Design review of the part built by this model. Coordinates are the model's own, in mm. Give positions to 0.01 mm unless a question says otherwise; leave off trailing zeros. Write each loop counter-clockwise with the first axis right and the second up, starting at its lowest first coordinate (ties: lowest second). Pieces come first, ordered by that corner, then holes. Notation, with made-up numbers: M 38,47.25 L 60,47.25 A18 cw 60,74.25 Z; hole C -24,54.25 d3. An arc over 180 degrees is marked long. Answer in a Markdown table with one row per item.
```python
from build123d import *

# Parameters (mm, degrees)
SKETCH1_W                      = 128
SKETCH1_H                      = 90
BOSS_EXTRUDE1_DEPTH            = 30
SKETCH4_R                      = 20
CUT_EXTRUDE3_DEPTH             = 84.791407674
F_15_0_15_DIAMETER_HOLE1_D     = 15
F_15_0_15_DIAMETER_HOLE1_DEPTH = 42
F_15_0_15_DIAMETER_HOLE1_TIP   = 4.506454643


with BuildPart() as part:
    # Sketch1 → Boss-Extrude1 (new body)
    with BuildSketch(Plane.XY):
        Rectangle(SKETCH1_W, SKETCH1_H)
    extrude(amount=BOSS_EXTRUDE1_DEPTH)

    # Sketch4 → Cut-Extrude3 (cut, through all)
    with BuildSketch(Plane.XY.offset(30)):
        with Locations((0, 10)):
            Circle(SKETCH4_R)
    extrude(amount=-CUT_EXTRUDE3_DEPTH, mode=Mode.SUBTRACT)

    # Ø15.0 (15) Diameter Hole1
    with Locations(Plane.XY.offset(30)):
        with Locations((-52, 19), (-52, -33), (52, -33), (52, 19)):
            Hole(F_15_0_15_DIAMETER_HOLE1_D / 2, depth=F_15_0_15_DIAMETER_HOLE1_DEPTH)
            with Locations((0, 0, -(F_15_0_15_DIAMETER_HOLE1_DEPTH + F_15_0_15_DIAMETER_HOLE1_TIP / 2))):  # 118° drill point
                Cone(0, F_15_0_15_DIAMETER_HOLE1_D / 2, F_15_0_15_DIAMETER_HOLE1_TIP, mode=Mode.SUBTRACT)


solid = part.part
```
1) Add section A-A (x = 52). Write out the cut boundary in (y, z), and give its area (3 significant figures).
Geometry says:
| item | result |
|---|---|
| outline | M -45,0 L -40.5,0 L -40.5,30 L -45,30 Z; M -25.5,0 L 11.5,0 L 11.5,30 L -25.5,30 Z; M 26.5,0 L 45,0 L 45,30 L 26.5,30 Z |
| area | 1,800 mm^2 |
2) To check wall thickness, follow probe 1 along Y at (x, z) = (52, 6); probe 2 along Y at (x, z) = (0, 17); probe 3 along Y at (x, z) = (-53, 5.75). State the ranges of each line that lie inside material, in increasing order. Write a range as [from, to].
Geometry says:
| item | result |
|---|---|
| probe 1 | [-45, -40.5], [-25.5, 11.5], [26.5, 45] |
| probe 2 | [-45, -10], [30, 45] |
| probe 3 | [-45, -40.43], [-25.57, 11.57], [26.43, 45] |
3) Add section D-D (y = -33). Write out the cut boundary in (x, z), and give its area (3 significant figures).
Geometry says:
| item | result |
|---|---|
| outline | M -64,0 L -59.5,0 L -59.5,30 L -64,30 Z; M -44.5,0 L 44.5,0 L 44.5,30 L -44.5,30 Z; M 59.5,0 L 64,0 L 64,30 L 59.5,30 Z |
| area | 2,940 mm^2 |
4) Add section B-B (z = 19.25). Write out the cut boundary in (x, y).
Geometry says:
| item | result |
|---|---|
| outline | M -64,-45 L 64,-45 L 64,45 L -64,45 Z; hole C -52,-33 d15; hole C -52,19 d15; hole C 0,10 d40; hole C 52,-33 d15; hole C 52,19 d15 |
5) Insertion check: P1, Ø17, axis at x = 52, y = 19, coming from the +Z side; P2, Ø3, axis at x = 5.5, y = 26, coming from the -Z side. Each pin has a flat end and moves straight along its axis. Give the tip position at first contact, or say it passes through.
Geometry says:
| item | result |
|---|---|
| P1 | z = 30 |
| P2 | through |
6) The part is to be moulded in two halves that separate along Y. For faces 1 (the face through (-51.024, 26.436, 14.79)), 2 (the face through (64, -1, 15)), 3 (the face through (-1, 45, 15)), say which applies: released by +Y, released by -Y, zero draft, split by the parting line, or undercut.
Geometry says:
| item | result |
|---|---|
| face 1 | undercut |
| face 2 | zero draft |
| face 3 | released by +Y |
7) Add section C-C (y = 10). Write out the cut boundary in (x, z), and give its area (3 significant figures).
Geometry says:
| item | result |
|---|---|
| outline | M -64,0 L -20,0 L -20,30 L -64,30 Z; M 20,0 L 64,0 L 64,30 L 20,30 Z |
| area | 2,640 mm^2 |
